Work out the finished part from the listing and answer in its coordinate system (mm). Face numbers are marked on the shaded views. A direction names the side the tool comes from. Round coordinates to 2 decimals unless told otherwise and drop trailing zeros. Write each loop counter-clockwise with the first axis right and the second up, starting at its lowest first coordinate (ties: lowest second). Pieces come first, ordered by that corner, then holes.
1. Flat-ended cylindrical pins translate along their axes: pin 1 Ø2 at (x, z) = (8.5, 0.5) entering from +Y; pin 2 Ø2 at (y, z) = (-1.5, 1.5) entering from +X; pin 3 Ø1.5 at (x, z) = (9, 4) entering from +Y; pin 4 Ø1.5 at (x, z) = (10, 4.5) entering from -Y. Find the tip coordinate at first contact, or state that the pin passes through.
2. Find section C-C (z = 4). Write down the section's boundary in (x, y).
3. Determine the mould class of the marked faces 4, 5 and 6 for opening direction X: pulls with the +X half, pulls with the -X half, needs draft (parallel to the pull), parting line crosses it, or undercut.
4. Find section D-D (x = 7). Write down the section's boundary in (y, z).
5. Find section B-B (y = -2.5). Write down the section's boundary in (x, z), and give its area (3 significant figures).
6. Find section A-A (z = 6). Write down the section's boundary in (x, y), and give its area (3 significant figures).
7. Straight lines are drawn through the part: probe 1 along X at (y, z) = (0, 8.5); probe 2 along Y at (x, z) = (11.35, 6); probe 3 along Z at (x, y) = (12.5, 1.25). For each, find the intervals that lie inside material, in ascending order.
8. A tool of negligible diameter and unlimited length cuts with its end or side. For the marked faces 1, 2 and 3, from which of +Z, -Z, +X, -X, +Y, -Y can it reach the whole face along a straight path? Write none if from no direction.
```python
from build123d import *

# Parameters (mm, degrees)
BOSS_EXTRUDE_1_DEPTH     = 2
SKETCH_3_R               = 0.5
BOSS_EXTRUDE_2_DEPTH     = 4
CUT_EXTRUDE_1_DEPTH      = 22.281643835
CUT_EXTRUDE_1_DEPTH_BACK = 22.281643835
SKETCH_4_W               = 2
SKETCH_4_H               = 8.093157612


with BuildPart() as part:
    # Sketch 1 → Boss-Extrude 1 (new body)
    with BuildSketch(Plane.XY):
        with BuildLine():
            Line((0, 2.25), (16.8, 2.25))
            ThreePointArc((16.8, 2.25), (19.05, 0), (16.8, -2.25))
            Line((16.8, -2.25), (0, -2.25))
            ThreePointArc((0, -2.25), (-2.25, 0), (0, 2.25))
        make_face()
    extrude(amount=BOSS_EXTRUDE_1_DEPTH)

    # Sketch 3 → Boss-Extrude 2 (add)
    with BuildSketch(Plane.ZY.offset(-12)):
        with BuildLine():
            Line((2, 2.25), (2, -2.249022682))
            Line((2, -2.249022682), (5.403845626, -2.939192745))
            ThreePointArc((5.403845626, -2.939192745), (8.999999942, 0.001391019), (5.403034747, 2.940982849))
            Line((5.403034747, 2.940982849), (2, 2.25))
        make_face()
        with Locations((5.99999997, 0.000977318)):
            Circle(SKETCH_3_R, mode=Mode.SUBTRACT)
    extrude(amount=BOSS_EXTRUDE_2_DEPTH)

    # Sketch 4 → Cut-Extrude 1 (cut, two sides: drawn at the far end of the back side and taken through both)
    with BuildSketch(Plane(origin=(0, 0, 0), x_dir=(1, 0, 0), z_dir=(0, 1, 0)).offset(-CUT_EXTRUDE_1_DEPTH_BACK)):
        with Locations((10, -6.046578806)):
            Rectangle(SKETCH_4_W, SKETCH_4_H)
    extrude(amount=CUT_EXTRUDE_1_DEPTH + CUT_EXTRUDE_1_DEPTH_BACK, mode=Mode.SUBTRACT)


solid = part.part
```
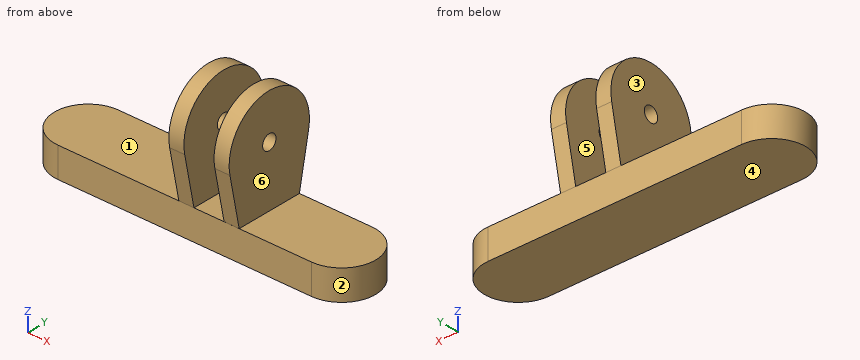
Worked answers:
1. pin 1: stops at y = 2.25
1. pin 2: stops at x = 18.99
1. pin 3: stops at y = 2.81
1. pin 4: passes through
2. outline: (8, -2.65) - (9, -2.65) - (9, 2.66) - (8, 2.66) - close; (11, -2.65) - (12, -2.65) - (12, 2.66) - (11, 2.66) - close
3. face 4: needs draft
3. face 5: undercut
3. face 6: pulls with the +X half
4. outline: (-2.25, 0) - (2.25, 0) - (2.25, 2) - (-2.25, 2) - close
5. outline: (8, 3.24) - (9, 3.24) - (9, 7.66) - (8, 7.66) - close; (11, 3.24) - (12, 3.24) - (12, 7.66) - (11, 7.66) - close
5. area: 8.84 mm2
6. outline: (8, -3) - (9, -3) - (9, -0.5) - (8, -0.5) - close; (8, 0.5) - (9, 0.5) - (9, 3) - (8, 3) - close; (11, -3) - (12, -3) - (12, -0.5) - (11, -0.5) - close; (11, 0.5) - (12, 0.5) - (12, 3) - (11, 3) - close
6. area: 10.0 mm2
7. probe 1: x = 8 to 9, 11 to 12
7. probe 2: y = -3 to -0.5, 0.5 to 3
7. probe 3: z = 0 to 2
8. face 1: +Z, +Y, -Y
8. face 2: +Z, -Z, +X
8. face 3: +Z, -X, +Y, -Y
